Geometry: final body of the model. Coordinates: model frame, mm. Coordinates: 2 decimals unless noted, no trailing zeros. Order: outer loops, then holes, each group sorted by start corner. A loop starts at its lowest first (then second) coordinate and runs counter-clockwise, first axis right, second up. Notation, with made-up numbers: M 38.5,-2.75 L 60.5,-2.75 A20 ccw 60.5,11.25 Z; hole C 23.25,-3 d11. An arc over 180 degrees is marked long. Write item = value, one per line.
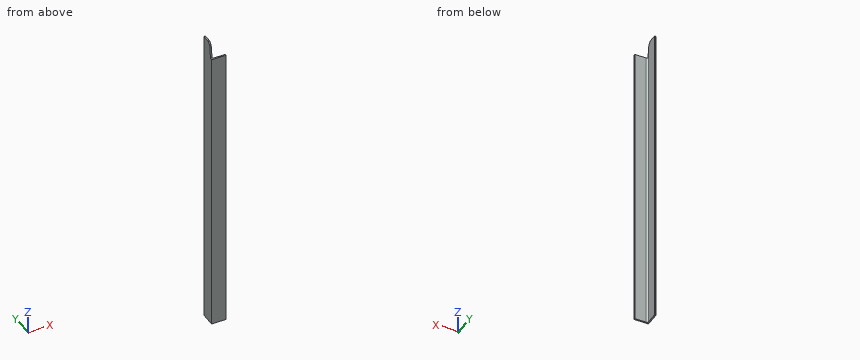
from build123d import *

# Parameters (mm, degrees)
GBT706_2008_050_5_1_DEPTH = 1073.5
CUT_EXTRUDE_1_REACH       = 1077.826


with BuildPart() as part:
    # Sketch1 → Gbt706-2008 热轧等边角钢 050×5(1) (new body)
    with BuildSketch(Plane.YX):
        with BuildLine():
            Line((0, 0), (0, 50))
            Line((0, 50), (3.333333333, 50))
            ThreePointArc((3.333333333, 50), (4.511844635, 49.511844635), (5, 48.333333333))
            Line((5, 48.333333333), (5, 10.5))
            ThreePointArc((5, 10.5), (6.610912703, 6.610912703), (10.5, 5))
            Line((10.5, 5), (48.333333333, 5))
            ThreePointArc((48.333333333, 5), (49.511844635, 4.511844635), (50, 3.333333333))
            Line((50, 3.333333333), (50, 0))
            Line((50, 0), (0, 0))
        make_face()
    extrude(amount=GBT706_2008_050_5_1_DEPTH)

    # 草图3 → 切除-拉伸1 (cut, up to next)
    with BuildSketch(Plane.ZY, mode=Mode.PRIVATE) as cut_extrude_1_sk1:
        Polygon((-56.5, 0), (-56.5, 7.501394609), (-52.022642316, 7.501394609), (-8.954715367, 12.028016136), (0, 21.973235089), (20, 21.973235089), (20, -8.026764911), (-56.5, -8.026764911), align=None)
    cut_extrude_1_tool1 = extrude(cut_extrude_1_sk1.sketch, amount=-CUT_EXTRUDE_1_REACH, mode=Mode.PRIVATE) & part.part
    add(cut_extrude_1_tool1.solids().sort_by_distance((0, 3.560964, -12.87534))[0], mode=Mode.SUBTRACT)


solid = part.part
1) Section B-B, the plane x = 26.5. Return loops of the section in (y, z).
Numbers:
outline = M 0,-1073.5 L 5,-1073.5 L 5,-56.5 L 0,-56.5 Z
2) Section A-A, the plane z = -867.5. Return loops of the section in (x, y), and give its area (3 significant figures).
Numbers:
outline = M 0,0 L 50,0 L 50,3.33 A1.67 ccw 48.33,5 L 10.5,5 A5.5 cw 5,10.5 L 5,48.33 A1.67 ccw 3.33,50 L 0,50 Z
area = 480 mm²
3) Pin query (flat end, axial travel): pin 1 (12 mm diameter, centred on x = 36, y = 12.5, fed in from +Z); pin 2 (10 mm diameter, centred on x = 28, z = -800.5, fed in from +Y); pin 3 (2.5 mm diameter, centred on x = 18, y = 5.5, fed in from +Z); pin 4 (5 mm diameter, centred on x = 2.5, z = -53.5, fed in from -Y). Return the tip coordinate at first contact, or that it passes through.
Numbers:
pin_1 = through
pin_2 = 5
pin_3 = -56.5
pin_4 = 7.5
4) Section C-C, the plane y = 33.5. Return loops of the section in (x, z).
Numbers:
outline = M 0,-1073.5 L 5,-1073.5 L 5,0 L 0,0 Z
5) Line query: L1, parallel to Y at x = 22, z = -304.5; L2, parallel to X at y = 7.5, z = -341. Output: solid intervals per line, ascending.
Numbers:
L1 = 0 to 5
L2 = 0 to 5.89
